from build123d import *

# Parameters (mm, degrees)
BASE_PLATE_DEPTH                = 12
EYE_BOSS_A_SKETCH_R             = 28
EYE_BOSS_A_56_DEPTH             = 14
EYE_HUB_A_SKETCH_R              = 28
EYE_HUB_A_56X4_DEPTH            = 4
EYE_WEB_A_DEPTH                 = 14
EYE_START                       = -14
EYE_BOSS_B_SKETCH_R             = 28
EYE_BOSS_B_DEPTH                = 14
EYE_HUB_B_SKETCH_R              = 28
EYE_HUB_B_56X4_DEPTH            = 4
SIDE_BOSS_SKETCH_R              = 25
SIDE_BOSS_50_DEPTH              = 62
SIDE_BOSS_FACE_CUT_A_SKETCH_R   = 25
SIDE_BOSS_FACE_CUT_A_50X8_DEPTH = 8
SIDE_BOSS_FACE_CUT_B_SKETCH_R   = 25
SIDE_BOSS_FACE_CUT_B_50X8_DEPTH = 8
SIDE_BORE_SKETCH_R              = 12.5
SIDE_BORE_25_DEPTH              = 46
EYE_BORE_SKETCH_R               = 16
EYE_BORE_32_DEPTH               = 80
CENTRAL_BODY_DEPTH              = 50
BODY_START                      = -50
BODY_SLOT_CUT_DEPTH             = 50
UPPER_LUG_A_SKETCH_R            = 18
UPPER_LUG_A_36_DEPTH            = 15
UPPER_LUG_B_SKETCH_R            = 18
UPPER_LUG_B_36_DEPTH            = 15
UPPER_CLEVIS_BODY_DEPTH         = 36
UPPER_CLEVIS_INFILL_SKETCH_W    = 18
UPPER_CLEVIS_INFILL_SKETCH_H    = 12
UPPER_CLEVIS_INFILL_DEPTH       = 36
CLEVIS_SLOT_A_SKETCH_W          = 36
CLEVIS_SLOT_A_SKETCH_H          = 18
CLEVIS_SLOT_A_DEPTH             = 12
CLEVIS_SLOT_B_SKETCH_W          = 36
CLEVIS_SLOT_B_SKETCH_H          = 18
CLEVIS_SLOT_B_DEPTH             = 12
LUG_PIN_HOLE_SKETCH_R           = 7.5
LUG_PIN_HOLE_15_DEPTH           = 60
SIDE_SLOT_CUT_DEPTH             = 60


with BuildPart() as part:
    # Base Plate Sketch → Base Plate (new body)
    with BuildSketch(Plane.XY):
        Polygon((0, 0), (14, 0), (48, 0), (62, 0), (62, 50), (0, 50), align=None)
    extrude(amount=BASE_PLATE_DEPTH)



with BuildPart() as body_2:
    # Eye Boss A Sketch → Eye Boss A _56 (new body)
    with BuildSketch(Plane(origin=(62, 0, 0), x_dir=(0, 0, -1), z_dir=(1, 0, 0))):
        with Locations((28, 25)):
            Circle(EYE_BOSS_A_SKETCH_R)
    extrude(amount=-EYE_BOSS_A_56_DEPTH)

    # Eye Hub A Sketch → Eye Hub A _56x4 (add)
    with BuildSketch(Plane(origin=(62, 0, 0), x_dir=(0, 0, -1), z_dir=(1, 0, 0))):
        with Locations((28, 25)):
            Circle(EYE_HUB_A_SKETCH_R)
    extrude(amount=EYE_HUB_A_56X4_DEPTH)


with BuildPart() as part_1:
    add(part.part)

    add(body_2.part)  # Eye Web A merges body 2
    # Eye Web A Sketch → Eye Web A (add)
    with BuildSketch(Plane(origin=(62, 0, 0), x_dir=(0, 0, -1), z_dir=(1, 0, 0))):
        with BuildLine():
            Line((15.390479787, 50), (0, 50))
            Line((0, 50), (0, 25.000000117))
            ThreePointArc((0, 25.000000117), (4.156064051, 39.678784639), (15.390479787, 50))
        make_face()
        with BuildLine():
            ThreePointArc((15.390479787, 0), (4.15606399, 10.32121546), (0, 25.000000117))
            Line((0, 25.000000117), (0, 0))
            Line((0, 0), (15.390479787, 0))
        make_face()
    extrude(amount=-EYE_WEB_A_DEPTH)

    # Eye Boss B Sketch → Eye Boss B (add)
    with BuildSketch(Plane.ZY.offset(EYE_START)):
        with Locations(Location((-28, 25, 0), (0, 0, 180))):
            Circle(EYE_BOSS_B_SKETCH_R)
        with BuildLine():
            Line((0, 25), (0, 50))
            Line((0, 50), (-15.390479787, 50))
            ThreePointArc((-15.390479787, 50), (-4.156064021, 39.678784589), (0, 25))
        make_face()
        with BuildLine():
            Line((0, 0), (0, 25))
            ThreePointArc((0, 25), (-4.156064021, 10.321215411), (-15.390479787, 0))
            Line((-15.390479787, 0), (0, 0))
        make_face()
    extrude(amount=EYE_BOSS_B_DEPTH)

    # Eye Hub B Sketch → Eye Hub B _56x4 (add)
    with BuildSketch(Plane.ZY):
        with Locations(Location((-28, 25, 0), (0, 0, 180))):
            Circle(EYE_HUB_B_SKETCH_R)
    extrude(amount=EYE_HUB_B_56X4_DEPTH)

    # Eye Bore Sketch → Eye Bore _32 (cut)
    with BuildSketch(Plane(origin=(66, 0, 0), x_dir=(0, 0, -1), z_dir=(1, 0, 0))):
        with Locations(Location((28, 25, 0), (0, 0, 180))):
            Circle(EYE_BORE_SKETCH_R)
    extrude(amount=-EYE_BORE_32_DEPTH, mode=Mode.SUBTRACT)



with BuildPart() as body_2_2:
    # Side Boss Sketch → Side Boss _50 (new body)
    with BuildSketch(Plane(origin=(62, 0, 0), x_dir=(0, 0, -1), z_dir=(1, 0, 0))):
        with Locations((-82, 25)):
            Circle(SIDE_BOSS_SKETCH_R)
    extrude(amount=-SIDE_BOSS_50_DEPTH)

    # Side Boss Face Cut A Sketch → Side Boss Face Cut A _50x8 (cut)
    with BuildSketch(Plane(origin=(62, 0, 0), x_dir=(0, 0, -1), z_dir=(1, 0, 0))):
        with Locations((-82, 25)):
            Circle(SIDE_BOSS_FACE_CUT_A_SKETCH_R)
    extrude(amount=-SIDE_BOSS_FACE_CUT_A_50X8_DEPTH, mode=Mode.SUBTRACT)

    # Side Boss Face Cut B Sketch → Side Boss Face Cut B _50x8 (cut)
    with BuildSketch(Plane.ZY):
        with Locations(Location((82, 25, 0), (0, 0, 180))):
            Circle(SIDE_BOSS_FACE_CUT_B_SKETCH_R)
    extrude(amount=-SIDE_BOSS_FACE_CUT_B_50X8_DEPTH, mode=Mode.SUBTRACT)

    # Side Bore Sketch → Side Bore _25 (cut)
    with BuildSketch(Plane.ZY.offset(-8)):
        with Locations((82, 25)):
            Circle(SIDE_BORE_SKETCH_R)
    extrude(amount=-SIDE_BORE_25_DEPTH, mode=Mode.SUBTRACT)


with BuildPart() as part_2:
    add(part_1.part)

    add(body_2_2.part)  # Central Body merges body 2 2
    # Central Body Sketch → Central Body (add)
    with BuildSketch(Plane(origin=(0, 50, 0), x_dir=(1, 0, 0), z_dir=(0, 1, 0))):
        Polygon((31, -12), (22, -12), (22, -71.244384349), (22, -85.354634245), (40, -85.354634245), (40, -71.244384349), (40, -12), align=None)
    extrude(amount=-CENTRAL_BODY_DEPTH)

    # Body Slot Sketch → Body Slot Cut (cut)
    with BuildSketch(Plane(origin=(40, 0, 0), x_dir=(0, 0, -1), z_dir=(1, 0, 0)).offset(BODY_START)):
        with BuildLine():
            Line((-85.354634245, 37.041446303), (-85.354634245, 12.958553697))
            ThreePointArc((-85.354634245, 12.958553697), (-69.5, 25), (-85.354634245, 37.041446303))
        make_face()
    extrude(amount=BODY_SLOT_CUT_DEPTH, mode=Mode.SUBTRACT)



with BuildPart() as body_2_3:
    # Upper Lug A Sketch → Upper Lug A _36 (new body)
    with BuildSketch(Plane.ZY.offset(-22)):
        with Locations((82, 110)):
            Circle(UPPER_LUG_A_SKETCH_R)
    extrude(amount=UPPER_LUG_A_36_DEPTH)


with BuildPart() as body_3:
    # Upper Lug B Sketch → Upper Lug B _36 (new body)
    with BuildSketch(Plane(origin=(40, 0, 0), x_dir=(0, 0, -1), z_dir=(1, 0, 0))):
        with Locations((-82, 110)):
            Circle(UPPER_LUG_B_SKETCH_R)
    extrude(amount=UPPER_LUG_B_36_DEPTH)


with BuildPart() as part_3:
    add(part_2.part)

    add(body_2_3.part)  # Upper Clevis Body merges body 2 3

    add(body_3.part)  # Upper Clevis Body merges body 3
    # Upper Clevis Profile Sketch → Upper Clevis Body (add)
    with BuildSketch(Plane.XY.offset(100)):
        Polygon((22, 62), (22, 49.773906214), (22, 25.080522604), (40, 25.080522604), (40, 50), (40, 62), (52, 62), (52, 92), (52, 106.982899018), (40, 106.982899018), (40, 76.982899018), (22, 76.982899018), (22, 106.982899018), (10, 106.982899018), (10, 92), (10, 62), align=None)
    extrude(amount=-UPPER_CLEVIS_BODY_DEPTH)

    # Upper Clevis Infill Sketch → Upper Clevis Infill (add)
    with BuildSketch(Plane.XY.offset(100)):
        with Locations((31, 82.982899018)):
            Rectangle(UPPER_CLEVIS_INFILL_SKETCH_W, UPPER_CLEVIS_INFILL_SKETCH_H)
    extrude(amount=-UPPER_CLEVIS_INFILL_DEPTH)

    # Clevis Slot A Sketch → Clevis Slot A (cut)
    with BuildSketch(Plane(origin=(52, 0, 0), x_dir=(0, 0, -1), z_dir=(1, 0, 0))):
        with Locations((-82, 71)):
            Rectangle(CLEVIS_SLOT_A_SKETCH_W, CLEVIS_SLOT_A_SKETCH_H)
    extrude(amount=-CLEVIS_SLOT_A_DEPTH, mode=Mode.SUBTRACT)

    # Clevis Slot B Sketch → Clevis Slot B (cut)
    with BuildSketch(Plane.ZY.offset(-10)):
        with Locations((82, 71)):
            Rectangle(CLEVIS_SLOT_B_SKETCH_W, CLEVIS_SLOT_B_SKETCH_H)
    extrude(amount=-CLEVIS_SLOT_B_DEPTH, mode=Mode.SUBTRACT)

    # Lug Pin Hole Sketch → Lug Pin Hole _15 (cut)
    with BuildSketch(Plane(origin=(55, 0, 0), x_dir=(0, 0, -1), z_dir=(1, 0, 0))):
        with Locations((-82, 110)):
            Circle(LUG_PIN_HOLE_SKETCH_R)
    extrude(amount=-LUG_PIN_HOLE_15_DEPTH, mode=Mode.SUBTRACT)

    # Side Slot Sketch → Side Slot Cut (cut)
    with BuildSketch(Plane.ZY.offset(-22)):
        with BuildLine():
            Line((69.5, 25), (94.5, 25))
            ThreePointArc((94.5, 25), (82, 37.5), (69.5, 25))
        make_face()
    extrude(amount=-SIDE_SLOT_CUT_DEPTH, mode=Mode.SUBTRACT)


solid = part_3.part
Verification items for the finished model (mm, model axes). A direction names the side the tool comes from. Coordinates: 2 decimals unless noted, no trailing zeros. Loops run counter-clockwise (first coordinate to the right, second up) from the corner with the lowest first, then second, coordinate; pieces in that order, holes last. Notation, with made-up numbers: M 82.5,7 L 100.5,7 A23 cw 100.5,19 Z; hole C 31,11.25 d10. An arc over 180 degrees is marked long. One line per item, written item: value.
1. Section check C-C on z = -2. Record the cut outline in (x, y).
Answers follow:
outline: M -4,14.61 L 0,14.61 L 0,0 L 14,0 L 14,50 L 0,50 L 0,35.39 L -4,35.39 Z; M 48,0 L 62,0 L 62,14.61 L 66,14.61 L 66,35.39 L 62,35.39 L 62,50 L 48,50 Z
2. Section check A-A on y = 110. Record the cut outline in (x, z), plus the area to 3 significant figures.
Answers follow:
outline: M 7,64 L 22,64 L 22,74.5 L 7,74.5 Z; M 7,89.5 L 22,89.5 L 22,100 L 7,100 Z; M 40,64 L 55,64 L 55,74.5 L 40,74.5 Z; M 40,89.5 L 55,89.5 L 55,100 L 40,100 Z
area: 630 mm^2
3. Gauge pin test, flat ends, axial feed: P1, Ø2, axis at x = 45, y = 37, coming from the -Z side; P2, Ø24, axis at y = 110, z = 82, coming from the -X side; P3, Ø8, axis at x = 47, z = -12.5, coming from the -Y side. Record the tip position at first contact, or that the pin passes through.
Answers follow:
P1: z = 0
P2: x = 7
P3: y = -0.47
4. Mould release check, pull along Y, two halves, no side actions. Record for faces 5 (the cylindrical face through (57.126, 34.736, -40.697)), 6 (the cylindrical face through (5.126, 43.237, -49.246)), 7 (the flat face through (11, 25, 12)): pulls with the +Y half, pulls with the -Y half, needs draft (parallel to the pull), parting line crosses it, or undercut.
Answers follow:
face 5: undercut
face 6: parting line crosses it
face 7: needs draft
5. Set-up check for faces 1 (the flat face through (40, 100, 82)), 2 (the flat face through (22, 41, 57)), 3 (the flat face through (62, 25, 4)), 4 (the flat face through (31, 50, 15)): record each of +Z, -Z, +X, -X, +Y, -Y from which the full face is reachable in a straight line by a thin tool's end or side.
Answers follow:
face 1: +Z, -Z, +Y
face 2: -X
face 3: +Z, +X
face 4: +X, -X, +Y
6. Material ranges on line 1 along Y through (x, z) = (48.5, 82); line 2 along Z through (x, y) = (42, 26); line 3 along Y through (x, z) = (14, 73.5), recorded low to high. Write a range as from..to.
Answers follow:
line 1: 0..12.5, 37.5..50, 80..102.5, 117.5..128
line 2: 0..12, 57.02..69.54, 94.46..106.98
line 3: 1.49..15.83, 34.17..48.51, 80..125.87
